Verification items for the finished model (mm, model axes). A direction names the side the tool comes from. Round coordinates to 2 decimals unless told otherwise and drop trailing zeros. Order: outer loops, then holes, each group sorted by start corner. A loop starts at its lowest first (then second) coordinate and runs counter-clockwise, first axis right, second up. Notation, with made-up numbers: M 13,18 L 71,18 A18 ccw 71,44 Z; hole C 25.25,-35 d7. An arc over 180 degrees is marked long. Use one line per item in the form item = value. Start each with the question number.
Item 1: Cross-section at C-C on x = -180. Enter the section's corners in (y, z), then the cut area to 3 significant figures.
Item 2: Cross-section at A-A on z = 12.5. Count the separate pieces of the cut face and the enclosed holes in it, then the cut area to 3 significant figures.
Item 3: Tool access check on faces 5 (the flat face through (-1, 47, 37)), 6 (the flat face through (340, -4, 20)). Record the directions out of +Z, -Z, +X, -X, +Y, -Y that give a thin tool (end or side, any length) a straight path to the whole face; none if there is none.
Item 4: Cross-section at B-B on y = 240. Enter the section's corners in (x, z).
Item 5: Thickness scan on probe 1 along Y at (x, z) = (0, 10); probe 2 along Y at (x, z) = (-180, 17); probe 3 along X at (y, z) = (85, 15.5). Record the ranges inside material, lowest first. Write a range as [from, to].
Item 6: Release check for a two-part mould opening along X. For faces 1 (the cylindrical face through (-334.297, -333.986, 20.28)), 2 (the flat face through (-4, 340, 20)), 3 (the cylindrical face through (-181.126, 188.576, 20.28)), 4 (the cylindrical face through (334.297, 333.986, 20.28)) record: +X half, -X half, draft (parallel to the pull), parting line (faces both ways), or undercut.
Item 7: Go/stop test with a flat-tipped pin: pin 1 Ø11.5 at (x, y) = (-60, -85) entering from +Z. Record where the tip stops, or that it passes through.
from build123d import *

# Parameters (mm, degrees)
SKETCH1_W           = 680
SKETCH1_H           = 680
BOSS_EXTRUDE1_DEPTH = 40
FILLET1_R           = 20
SKETCH2_W           = 155
SKETCH2_H           = 205
SKETCH2_R           = 5.05
CUT_EXTRUDE1_DEPTH  = 3
SKETCH3_R           = 5.05
CUT_EXTRUDE2_DEPTH  = 219
SKETCH4_R           = 45
CUT_EXTRUDE3_DEPTH  = 219
SKETCH5_R           = 8.65
CUT_EXTRUDE4_DEPTH  = 219
SKETCH6_R           = 4.2
CUT_EXTRUDE5_DEPTH  = 219
SKETCH7_R           = 25
CUT_EXTRUDE6_DEPTH  = 219


with BuildPart() as part:
    # Sketch1 → Boss-Extrude1 (new body)
    with BuildSketch(Plane.XY):
        Rectangle(SKETCH1_W, SKETCH1_H)
    extrude(amount=BOSS_EXTRUDE1_DEPTH)

    # Fillet1
    fillet1_edges = [part.edges().sort_by_distance(p)[0] for p in [
        (-340, 340, 20),
        (340, 340, 20),
        (340, -340, 20),
        (-340, -340, 20),
    ]]
    fillet(fillet1_edges, radius=FILLET1_R)

    # Sketch2 → Cut-Extrude1 (cut)
    with BuildSketch(Plane.XY.offset(40)):
        Rectangle(SKETCH2_W, SKETCH2_H)
        with Locations((-60, 85)):
            Circle(SKETCH2_R, mode=Mode.SUBTRACT)
        with Locations((-20, 85)):
            Circle(SKETCH2_R, mode=Mode.SUBTRACT)
        with Locations((20, 85)):
            Circle(SKETCH2_R, mode=Mode.SUBTRACT)
        with Locations((60, 85)):
            Circle(SKETCH2_R, mode=Mode.SUBTRACT)
        with Locations(Location((60, -85, 0), (0, 0, 180))):
            Circle(SKETCH2_R, mode=Mode.SUBTRACT)
        with Locations(Location((20, -85, 0), (0, 0, 180))):
            Circle(SKETCH2_R, mode=Mode.SUBTRACT)
        with Locations(Location((-20, -85, 0), (0, 0, 180))):
            Circle(SKETCH2_R, mode=Mode.SUBTRACT)
        with Locations(Location((-60, -85, 0), (0, 0, 180))):
            Circle(SKETCH2_R, mode=Mode.SUBTRACT)
    extrude(amount=-CUT_EXTRUDE1_DEPTH, mode=Mode.SUBTRACT)

    # Sketch3 → Cut-Extrude2 (cut)
    with BuildSketch(Plane.XY.offset(40)):
        with Locations(Location((-60, 85, 0), (0, 0, 180))):
            Circle(SKETCH3_R)
        with Locations(Location((-60, -85, 0), (0, 0, 180))):
            Circle(SKETCH3_R)
        with Locations(Location((-20, -85, 0), (0, 0, 180))):
            Circle(SKETCH3_R)
        with Locations(Location((60, -85, 0), (0, 0, 180))):
            Circle(SKETCH3_R)
        with Locations(Location((60, 85, 0), (0, 0, 180))):
            Circle(SKETCH3_R)
        with Locations(Location((20, 85, 0), (0, 0, 180))):
            Circle(SKETCH3_R)
        with Locations(Location((-20, 85, 0), (0, 0, 180))):
            Circle(SKETCH3_R)
    extrude(amount=-CUT_EXTRUDE2_DEPTH, mode=Mode.SUBTRACT)

    # Sketch4 → Cut-Extrude3 (cut)
    with BuildSketch(Plane.XY.offset(37)):
        Circle(SKETCH4_R)
    extrude(amount=-CUT_EXTRUDE3_DEPTH, mode=Mode.SUBTRACT)

    # Sketch5 → Cut-Extrude4 (cut)
    with BuildSketch(Plane.XY.offset(40)):
        with Locations((-180, 180)):
            Circle(SKETCH5_R)
        with Locations((180, 180)):
            Circle(SKETCH5_R)
        with Locations((180, -180)):
            Circle(SKETCH5_R)
        with Locations((-180, -180)):
            Circle(SKETCH5_R)
    extrude(amount=-CUT_EXTRUDE4_DEPTH, mode=Mode.SUBTRACT)

    # Sketch6 → Cut-Extrude5 (cut)
    with BuildSketch(Plane.XY.offset(40)):
        with Locations((0, -313)):
            Circle(SKETCH6_R)
        with Locations((45.899346401, -233.5)):
            Circle(SKETCH6_R)
        with Locations((-45.899346401, -233.5)):
            Circle(SKETCH6_R)
    extrude(amount=-CUT_EXTRUDE5_DEPTH, mode=Mode.SUBTRACT)

    # Sketch7 → Cut-Extrude6 (cut)
    with BuildSketch(Plane.XY.offset(40)):
        with Locations((-240, 240)):
            Circle(SKETCH7_R)
        with Locations((240, 240)):
            Circle(SKETCH7_R)
        with Locations((240, -240)):
            Circle(SKETCH7_R)
        with Locations((-240, -240)):
            Circle(SKETCH7_R)
    extrude(amount=-CUT_EXTRUDE6_DEPTH, mode=Mode.SUBTRACT)


solid = part.part
Output values:
q1.outline = M -340,0 L -188.65,0 L -188.65,40 L -340,40 Z; M -171.35,0 L 171.35,0 L 171.35,40 L -171.35,40 Z; M 188.65,0 L 340,0 L 340,40 L 188.65,40 Z
q1.area = 25,800 mm2
q2.separate_pieces = 1
q2.enclosed_holes = 19
q2.area = 446,000 mm2
q3.face_5 = +Z
q3.face_6 = +Z, -Z, +X, +Y, -Y
q4.outline = M -340,0 L -265,0 L -265,40 L -340,40 Z; M -215,0 L 215,0 L 215,40 L -215,40 Z; M 265,0 L 340,0 L 340,40 L 265,40 Z
q5.probe_1 = [-340, -317.2], [-308.8, -45], [45, 340]
q5.probe_2 = [-340, -188.65], [-171.35, 171.35], [188.65, 340]
q5.probe_3 = [-340, -65.05], [-54.95, -25.05], [-14.95, 14.95], [25.05, 54.95], [65.05, 340]
q6.face_1 = -X half
q6.face_2 = draft
q6.face_3 = undercut
q6.face_4 = +X half
q7.pin_1 = 37
